The listing builds one solid part. Answer for the finished solid, in the listing's coordinates (mm). Give positions to 0.01 mm unless a question says otherwise; leave off trailing zeros. Order: outer loops, then holes, each group sorted by start corner. A loop starts at its lowest first (then second) coordinate and runs counter-clockwise, first axis right, second up. Notation, with made-up numbers: (88, -13) - (130, -13) arc R6 cw to (130, -3) - close; hole circle Ø5 at (71.5, -5.75). An arc over 180 degrees is marked (long way). Answer in a Markdown table with one row per item.
from build123d import *

# Parameters (mm, degrees)
M100_CLEARANCE_HOLE1_D       = 110
M100_CLEARANCE_HOLE1_DEPTH   = 48.300542714
M100_CLEARANCE_HOLE1_TIP     = 157.142859071
F_8_0_8_DIAMETER_HOLE1_D     = 8
F_8_0_8_DIAMETER_HOLE1_DEPTH = 140.145647392
FILLET1_R                    = 5


with BuildPart() as part:
    # Sketch1 → Revolve1 (revolve)
    with BuildSketch(Plane(origin=(0, 234.743963655, 0), x_dir=(1, 0, 0), z_dir=(0, 1, 0))):
        Polygon((551.230642584, 1664.998443067), (521.230642584, 1664.998443067), (521.230642584, 1514.998443067), (586.230642584, 1514.998443067), (586.230642584, 1564.998443067), align=None)
    revolve(axis=Axis((521.230642584, 234.743963655, -1664.998443067), (0, 0, 1)))

    # M100 clearance hole1
    with Locations(Plane.XY.offset(-1514.998443067)):
        with Locations((521.230642584, 234.743963655)):
            Hole(M100_CLEARANCE_HOLE1_D / 2, depth=M100_CLEARANCE_HOLE1_DEPTH)
            with Locations((0, 0, -(M100_CLEARANCE_HOLE1_DEPTH + M100_CLEARANCE_HOLE1_TIP / 2))):  # 38.580092° drill point
                Cone(0, M100_CLEARANCE_HOLE1_D / 2, M100_CLEARANCE_HOLE1_TIP, mode=Mode.SUBTRACT)

    # Ø8.0 (8) diameter hole1
    with Locations(Plane(origin=(558.630703666, 287.906313406, -1524.998443067), x_dir=(0.817882303865, -0.575385555106, 0), z_dir=(0.575385555106, 0.817882303865, 0))):
        with Locations((0, 0)):
            Hole(F_8_0_8_DIAMETER_HOLE1_D / 2, depth=F_8_0_8_DIAMETER_HOLE1_DEPTH)

    # Fillet1
    fillet1_edges = [part.edges().sort_by_distance(p)[0] for p in [
        (491.230642584, 234.743963655, -1664.998443067),
    ]]
    fillet(fillet1_edges, radius=FILLET1_R)


solid = part.part
Item 1: Each of these flat-tipped pins is pushed along its axis until it touches: P1, Ø1, axis at x = 534, y = 262.5, coming from the -Z side; P2, Ø8, axis at y = 201, z = -1627.5, coming from the -X side; P3, Ø10, axis at y = 251.5, z = -1646.5, coming from the +X side. Where does it stop, or does it pass through?
Answer block:
| item | result |
|---|---|
| P1 | z = -1663.47 |
| P2 | x = 489.54 |
| P3 | x = 556.55 |
Item 2: Consider line 1 (Y direction, x = 506.5, z = -1629); line 2 (Y direction, x = 517.5, z = -1630); line 3 (X direction, y = 221, z = -1626). Determine where each line is inside the solid, lowest interval first.
Answer block:
| item | result |
|---|---|
| line 1 | 194.77 to 206.33, 263.16 to 274.72 |
| line 2 | 192.66 to 203.31, 266.18 to 276.83 |
| line 3 | 479.8 to 491.17, 551.29 to 562.66 |
Item 3: Find section A-A on z = -1593. Write down the section's boundary in (x, y).
Answer block:
| item | result |
|---|---|
| outline | circle Ø110.4 at (521.23, 234.74); hole circle Ø89.21 at (521.23, 234.74) |
Item 4: Find section B-B on z = -1647.5. Write down the section's boundary in (x, y).
Answer block:
| item | result |
|---|---|
| outline | circle Ø72.25 at (521.23, 234.74); hole circle Ø51.06 at (521.23, 234.74) |
Item 5: Determine the mould class of faces 1 (the face through (470.425, 213.679, -1539.487)), 2 (the face through (507.1, 171.3, -1540.3)), 3 (the face through (574.5, 249.5, -1514.998)), 4 (the face through (487.135, 185.373, -1528.964)) for opening direction Y: pulls with the +Y half, pulls with the -Y half, needs draft (parallel to the pull), parting line crosses it, or undercut.
Answer block:
| item | result |
|---|---|
| face 1 | undercut |
| face 2 | parting line crosses it |
| face 3 | needs draft |
| face 4 | undercut |
